Geometry check sheet. Reference: the model listing, model coordinates, mm. Face numbers are marked on the shaded views. A direction names the side the tool comes from. Round coordinates to 2 decimals unless told otherwise and drop trailing zeros. Order: outer loops, then holes, each group sorted by start corner. A loop starts at its lowest first (then second) coordinate and runs counter-clockwise, first axis right, second up.
(1) Cross-section at B-B on x = 11.25. Enter the section's corners in (y, z), and give its area (3 significant figures).
(2) Cross-section at C-C on z = 23.75. Enter the section's corners in (x, y), and give its area (3 significant figures).
(3) Gauge pin test, flat ends, axial feed: P1, Ø3, axis at y = 26, z = 5.5, coming from the +X side; P2, Ø11.5, axis at x = 11.25, z = 12.5, coming from the +Y side; P3, Ø8, axis at y = 24.5, z = 22, coming from the -X side; P4, Ø11, axis at x = 35, y = 17, coming from the -Z side. Record the tip position at first contact, or that the pin passes through.
(4) Set-up check for the marked faces 4, 5 and 6: record each of +Z, -Z, +X, -X, +Y, -Y from which the full face is reachable in a straight line by a thin tool's end or side.
(5) Thickness scan on L1, parallel to X at y = 9.75, z = 12.5; L2, parallel to X at y = 25.5, z = 6; L3, parallel to X at y = 3.5, z = 12.5. Record the ranges inside material, lowest first.
(6) Draft check along X on the marked faces 1, 2 and 3. Enter one of: pulls with the +X half, pulls with the -X half, needs draft (parallel to the pull), parting line crosses it, or undercut.
(7) Cross-section at A-A on y = 17. Enter the section's corners in (x, z), and give its area (3 significant figures).
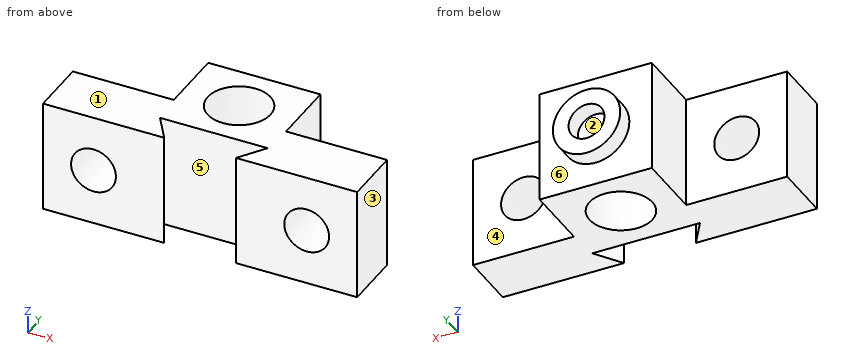
from build123d import *

# Parameters (mm, degrees)
STEPPED_BLOCK_DEPTH          = 25
CROSS_HOLE_SKETCH_R          = 7
CROSS_HOLE_11_DEPTH          = 25
STEP_HOLES_SKETCH_R          = 5
STEP_HOLES_2X_DEPTH_13_DEPTH = 13
TOP_BOSS_SKETCH_R            = 7.5
TOP_BOSS_DEPTH               = 4
TOP_BOSS_BORE_SKETCH_R       = 4
TOP_BOSS_BORE_DEPTH          = 4


with BuildPart() as part:
    # Stepped Block Profile → Stepped Block (new body)
    with BuildSketch(Plane.XY):
        Polygon((0, 0), (0, 13), (22.5, 13), (22.5, 28), (35, 28), (47.5, 28), (47.5, 13), (70, 13), (70, 0), (43, 0), (47, 6), (35, 6), (23, 6), (27, 0), align=None)
    extrude(amount=STEPPED_BLOCK_DEPTH)

    # Cross Hole Sketch → Cross Hole Ø11 (cut)
    with BuildSketch(Plane.XY.offset(25)):
        with Locations((35, 17)):
            Circle(CROSS_HOLE_SKETCH_R)
    extrude(amount=-CROSS_HOLE_11_DEPTH, mode=Mode.SUBTRACT)

    # Step Holes Sketch → Step Holes 2x Depth 13 (cut)
    with BuildSketch(Plane(origin=(0, 13, 0), x_dir=(1, 0, 0), z_dir=(0, 1, 0))):
        with Locations(Location((58.75, -12.5, 0), (0, 0, 270))):
            Circle(STEP_HOLES_SKETCH_R)
        with Locations(Location((11.25, -12.5, 0), (0, 0, 270))):
            Circle(STEP_HOLES_SKETCH_R)
    extrude(amount=-STEP_HOLES_2X_DEPTH_13_DEPTH, mode=Mode.SUBTRACT)

    # Top Boss Sketch → Top Boss (add)
    with BuildSketch(Plane(origin=(0, 28, 0), x_dir=(1, 0, 0), z_dir=(0, 1, 0))):
        with Locations(Location((35, -12.5, 0), (0, 0, 270))):
            Circle(TOP_BOSS_SKETCH_R)
    extrude(amount=TOP_BOSS_DEPTH)

    # Top Boss Bore Sketch → Top Boss Bore (cut)
    with BuildSketch(Plane(origin=(0, 32, 0), x_dir=(1, 0, 0), z_dir=(0, 1, 0))):
        with Locations(Location((35, -12.5, 0), (0, 0, 270))):
            Circle(TOP_BOSS_BORE_SKETCH_R)
    extrude(amount=-TOP_BOSS_BORE_DEPTH, mode=Mode.SUBTRACT)


solid = part.part
Found:
1. outline: (0, 0) - (13, 0) - (13, 7.5) - (0, 7.5) - close; (0, 17.5) - (13, 17.5) - (13, 25) - (0, 25) - close
1. area: 195 mm2
2. outline: (0, 0) - (27, 0) - (23, 6) - (47, 6) - (43, 0) - (70, 0) - (70, 13) - (47.5, 13) - (47.5, 28) - (22.5, 28) - (22.5, 13) - (0, 13) - close; hole circle Ø14 at (35, 17)
2. area: 1,010 mm2
3. P1: stops at x = 47.5
3. P2: stops at y = 13
3. P3: stops at x = 22.5
3. P4: passes through
4. face 4: +Z, -Z, +X, +Y
4. face 5: +Z, -Z
4. face 6: +Y
5. L1: x = 0 to 6.25, 16.25 to 53.75, 63.75 to 70
5. L2: x = 22.5 to 47.5
5. L3: x = 0 to 6.25, 16.25 to 24.67, 45.33 to 53.75, 63.75 to 70
6. face 1: needs draft
6. face 2: undercut
6. face 3: pulls with the +X half
7. outline: (22.5, 0) - (28, 0) - (28, 25) - (22.5, 25) - close; (42, 0) - (47.5, 0) - (47.5, 25) - (42, 25) - close
7. area: 275 mm2
